```python
from build123d import *

# Parameters (mm, degrees)
SKETCH2_R           = 7
BOSS_EXTRUDE1_DEPTH = 10


with BuildPart() as part:
    # Sketch2 → Boss-Extrude1 (new body)
    with BuildSketch(Plane(origin=(0, 0, 0), x_dir=(1, 0, 0), z_dir=(0, 1, 0))):
        with BuildLine():
            Line((65, -20), (-65, -20))
            ThreePointArc((-65, -20), (-68.535533906, -18.535533906), (-70, -15))
            Line((-70, -15), (-70, 15))
            ThreePointArc((-70, 15), (-68.535533906, 18.535533906), (-65, 20))
            Line((-65, 20), (65, 20))
            ThreePointArc((65, 20), (68.535533906, 18.535533906), (70, 15))
            Line((70, 15), (70, -15))
            ThreePointArc((70, -15), (68.535533906, -18.535533906), (65, -20))
        make_face()
        with Locations(Location((-55, 0, 0), (0, 0, 270))):
            Circle(SKETCH2_R, mode=Mode.SUBTRACT)
        with Locations(Location((55, 0, 0), (0, 0, 90))):
            Circle(SKETCH2_R, mode=Mode.SUBTRACT)
    extrude(amount=BOSS_EXTRUDE1_DEPTH)


solid = part.part
```
Geometry check sheet. Reference: the model listing, model coordinates, mm. Coordinates: 2 decimals unless noted, no trailing zeros. Loops run counter-clockwise (first coordinate to the right, second up) from the corner with the lowest first, then second, coordinate; pieces in that order, holes last. Notation, with made-up numbers: (-17, 48) -> (-8, 48) arc R24 ccw to (-8, 77) -> close; hole circle Ø11 at (2, 31.25). An arc over 180 degrees is marked (long way). Put each result on its own line as item: value.
1) Thickness scan on line 1 (X direction, y = 2, z = 0); line 2 (Z direction, x = 55, y = 4.25); line 3 (X direction, y = 6.5, z = -15.5). Record the ranges inside material, lowest first.
Result set:
line 1: x = -70 to -62, -48 to 48, 62 to 70
line 2: z = -20 to -7, 7 to 20
line 3: x = -69.97 to 69.97
2) Gauge pin test, flat end, axial feed: pin 1 Ø12.5 at (x, z) = (55, 0) entering from -Y. Record the tip position at first contact, or that the pin passes through.
Result set:
pin 1: passes through
3) Cross-section at A-A on y = 7.75. Record the boundary of the cut face in (x, z).
Result set:
outline: (-70, -15) arc R5 ccw to (-65, -20) -> (65, -20) arc R5 ccw to (70, -15) -> (70, 15) arc R5 ccw to (65, 20) -> (-65, 20) arc R5 ccw to (-70, 15) -> close; hole circle Ø14 at (-55, 0); hole circle Ø14 at (55, 0)
4) Cross-section at B-B on z = 0. Record the boundary of the cut face in (x, y), plus the area to 3 significant figures.
Result set:
outline: (-70, 0) -> (-62, 0) -> (-62, 10) -> (-70, 10) -> close; (-48, 0) -> (48, 0) -> (48, 10) -> (-48, 10) -> close; (62, 0) -> (70, 0) -> (70, 10) -> (62, 10) -> close
area: 1,120 mm^2
5) Cross-section at C-C on x = 55. Record the boundary of the cut face in (y, z), plus the area to 3 significant figures.
Result set:
outline: (0, -20) -> (10, -20) -> (10, -7) -> (0, -7) -> close; (0, 7) -> (10, 7) -> (10, 20) -> (0, 20) -> close
area: 260 mm^2
6) Release check for a two-part mould opening along X. For faces 1 (the cylindrical face through (48.06, 4.93, 0.91)), 2 (the flat face through (1, 10, 0)), 3 (the cylindrical face through (-68, 5, 19)), 4 (the cylindrical face through (-48.06, 4.93, -0.91)) record: released by +X, released by -X, zero draft, split by the parting line, or undercut.
Result set:
face 1: undercut
face 2: zero draft
face 3: released by -X
face 4: undercut
